Design review of the part built by this model. Coordinates are the model's own, in mm. Give positions to 0.01 mm unless a question says otherwise; leave off trailing zeros. Loops run counter-clockwise (first coordinate to the right, second up) from the corner with the lowest first, then second, coordinate; pieces in that order, holes last. Notation, with made-up numbers: (77.5, 88) -> (125.5, 88) arc R27 cw to (125.5, 107) -> close; hole circle Ø6 at (30, -0.75). An arc over 180 degrees is marked (long way). Use a Markdown table: item, result. Add a question column.
1. Add section B-B (y = 0). State the section outline as (x, z) points, and give its area (3 significant figures).
2. For pin 1 Ø2.5 at (x, y) = (60, 0) entering from +Z, flat-tipped, find the tip position at first contact; note if it passes through.
3. Draft analysis for pull direction Y (two halves, no side actions). For faces 1 (the flat face through (-75, -1, 0)), 2 (the flat face through (-1, 91.5, 0)), 3 (the flat face through (-1, -91.5, 0)), 4 (the cylindrical face through (-61.94, -0.8, -0.06)), state which applies: pulls with the +Y half, pulls with the -Y half, needs draft (parallel to the pull), parting line crosses it, or undercut.
4. Add section A-A (x = 0). State the section outline as (y, z) points, and give its area (3 significant figures).
5. To check wall thickness, follow line 1 (Y direction, x = -60, z = 1.25). State the ranges of the line that lie inside material, in increasing order.
```python
from build123d import *

# Parameters (mm, degrees)
SKETCH1_W           = 150
SKETCH1_H           = 183
BOSS_EXTRUDE1_DEPTH = 4
M5_TAPPED_HOLE1_D   = 4.2


with BuildPart() as part:
    # Sketch1 → Boss-Extrude1 (new, symmetric)
    with BuildSketch(Plane.XY):
        Rectangle(SKETCH1_W, SKETCH1_H)
    extrude(amount=BOSS_EXTRUDE1_DEPTH, both=True)

    # M5 Tapped Hole1 (through all)
    with Locations(Plane.XY.offset(4)):
        with Locations((-60, 0), (0, 0), (60, 0)):
            Hole(M5_TAPPED_HOLE1_D / 2)


solid = part.part
```
Taken from the geometry:
| question | item | result |
|---|---|---|
| 1 | outline | (-75, -4) -> (-62.1, -4) -> (-62.1, 4) -> (-75, 4) -> close; (-57.9, -4) -> (-2.1, -4) -> (-2.1, 4) -> (-57.9, 4) -> close; (2.1, -4) -> (57.9, -4) -> (57.9, 4) -> (2.1, 4) -> close; (62.1, -4) -> (75, -4) -> (75, 4) -> (62.1, 4) -> close |
| 1 | area | 1,100 mm^2 |
| 2 | pin 1 | passes through |
| 3 | face 1 | needs draft |
| 3 | face 2 | pulls with the +Y half |
| 3 | face 3 | pulls with the -Y half |
| 3 | face 4 | undercut |
| 4 | outline | (-91.5, -4) -> (-2.1, -4) -> (-2.1, 4) -> (-91.5, 4) -> close; (2.1, -4) -> (91.5, -4) -> (91.5, 4) -> (2.1, 4) -> close |
| 4 | area | 1,430 mm^2 |
| 5 | line 1 | y = -91.5 to -2.1, 2.1 to 91.5 |
